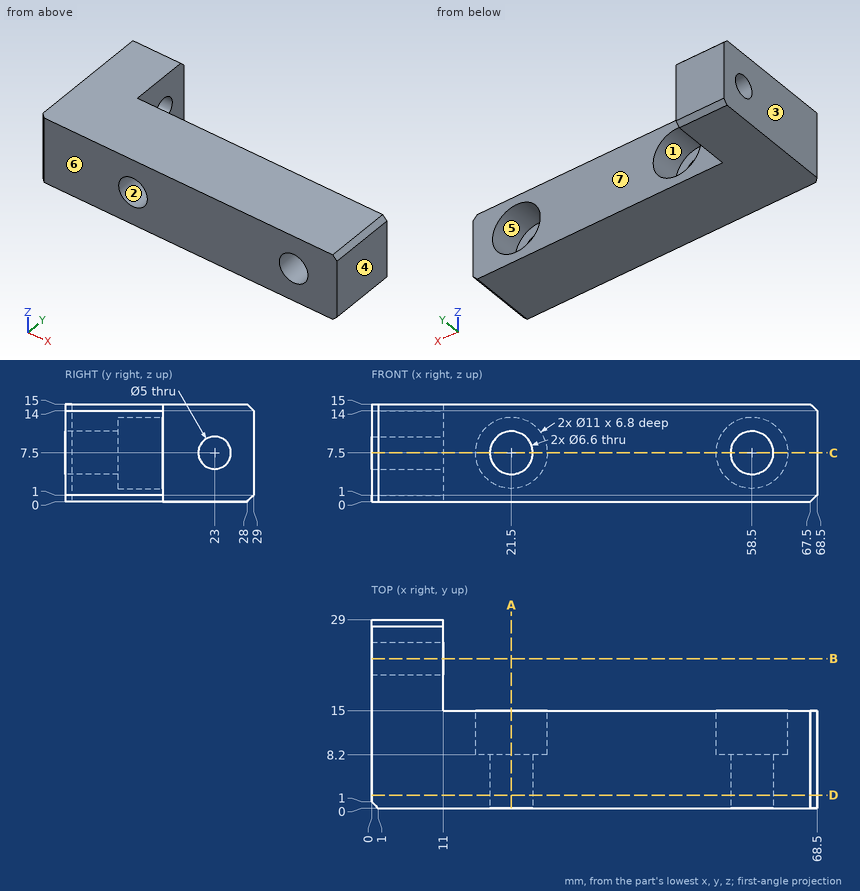
For this review, use the dimensioned drawing (mm, ordinates from the lowest corner) and the shaded views. A direction names the side the tool comes from. Round coordinates to 2 decimals unless told otherwise and drop trailing zeros. Write each loop counter-clockwise with the first axis right and the second up, starting at its lowest first coordinate (ties: lowest second). Pieces come first, ordered by that corner, then holes. Notation, with made-up numbers: (4, 24.25) -> (49, 24.25) arc R23 ccw to (49, 58.25) -> close; hole circle Ø3 at (68.5, 18). An arc over 180 degrees is marked (long way). Use CSV: the item, a comma, the result in double quotes.
(1) Clearance check with flat-ended pins moving along their axes: P1, Ø6, axis at x = 58.5, z = 7.5, coming from the +Y side; P2, Ø4.5, axis at x = 36, z = 8, coming from the +Y side; P3, Ø1, axis at y = 18.5, z = 4, coming from the +X side. State where each tip first meets the part, or that it passes through.
Computed values:
P1,"through"
P2,"y = 15"
P3,"x = 11"
(2) Draft analysis for pull direction X (two halves, no side actions). For the marked faces 1, 2, 3 and 4, state which applies: +X half, -X half, draft (parallel to the pull), parting line (faces both ways), or undercut.
Computed values:
face 1,"undercut"
face 2,"undercut"
face 3,"-X half"
face 4,"+X half"
(3) Consider section D-D, the plane y = 2. Give the boundary of the cut face in (x, z), plus the area to 3 significant figures.
Computed values:
outline,"(0, 0) -> (67.5, 0) -> (68.5, 1) -> (68.5, 14) -> (67.5, 15) -> (0, 15) -> close; hole circle Ø6.6 at (21.5, 7.5); hole circle Ø6.6 at (58.5, 7.5)"
area,"958 mm²"
(4) Consider section A-A, the plane x = 21.5. Give the boundary of the cut face in (y, z).
Computed values:
outline,"(0, 0) -> (15, 0) -> (15, 2) -> (8.2, 2) -> (8.2, 4.2) -> (0, 4.2) -> close; (0, 10.8) -> (8.2, 10.8) -> (8.2, 13) -> (15, 13) -> (15, 15) -> (0, 15) -> close"
(5) To check wall thickness, follow L1, parallel to X at y = 10, z = 7.25; L2, parallel to Z at x = 58.5, y = 2; L3, parallel to X at y = 9.5, z = 8.75. State the ranges of each line that lie inside material, in increasing order. Write a range as [from, to].
Computed values:
L1,"[0, 16.01], [26.99, 53.01], [63.99, 68.5]"
L2,"[0, 4.2], [10.8, 15]"
L3,"[0, 16.14], [26.86, 53.14], [63.86, 68.5]"
(6) Consider section C-C, the plane z = 7.5. Give the boundary of the cut face in (x, y).
Computed values:
outline,"(0, 1) -> (1, 0) -> (18.2, 0) -> (18.2, 8.2) -> (16, 8.2) -> (16, 15) -> (11, 15) -> (11, 20.5) -> (0, 20.5) -> close; (0, 25.5) -> (11, 25.5) -> (11, 29) -> (0, 29) -> close; (24.8, 0) -> (55.2, 0) -> (55.2, 8.2) -> (53, 8.2) -> (53, 15) -> (27, 15) -> (27, 8.2) -> (24.8, 8.2) -> close; (61.8, 0) -> (68.5, 0) -> (68.5, 15) -> (64, 15) -> (64, 8.2) -> (61.8, 8.2) -> close"
(7) Consider section B-B, the plane y = 23. Give the boundary of the cut face in (x, z).
Computed values:
outline,"(0, 0) -> (11, 0) -> (11, 5) -> (0, 5) -> close; (0, 10) -> (11, 10) -> (11, 15) -> (0, 15) -> close"
(8) For the marked faces 5, 6 and 7, list the 3-axis set-ups (+Z, -Z, +X, -X, +Y, -Y) from which the entire face can be reached by the end or side of a thin tool; tool diameter is ignored.
Computed values:
face 5,"+Y"
face 6,"+Z, -Z, +X, -X, -Y"
face 7,"+Z, -Z, +X, +Y"
